Source: three-view drawing plus pictorial views. Frame: mm from the lowest corner of the part. A direction names the side the tool comes from. Give positions to 0.01 mm unless a question says otherwise; leave off trailing zeros. Loops run counter-clockwise (first coordinate to the right, second up) from the corner with the lowest first, then second, coordinate; pieces in that order, holes last. Notation, with made-up numbers: (23.25, -33) - (63.25, -33) arc R29 ccw to (63.25, -8) - close; hole circle Ø7 at (-30, -7.75). An arc over 180 degrees is marked (long way). Answer as a JSON object with one key per item and string values.
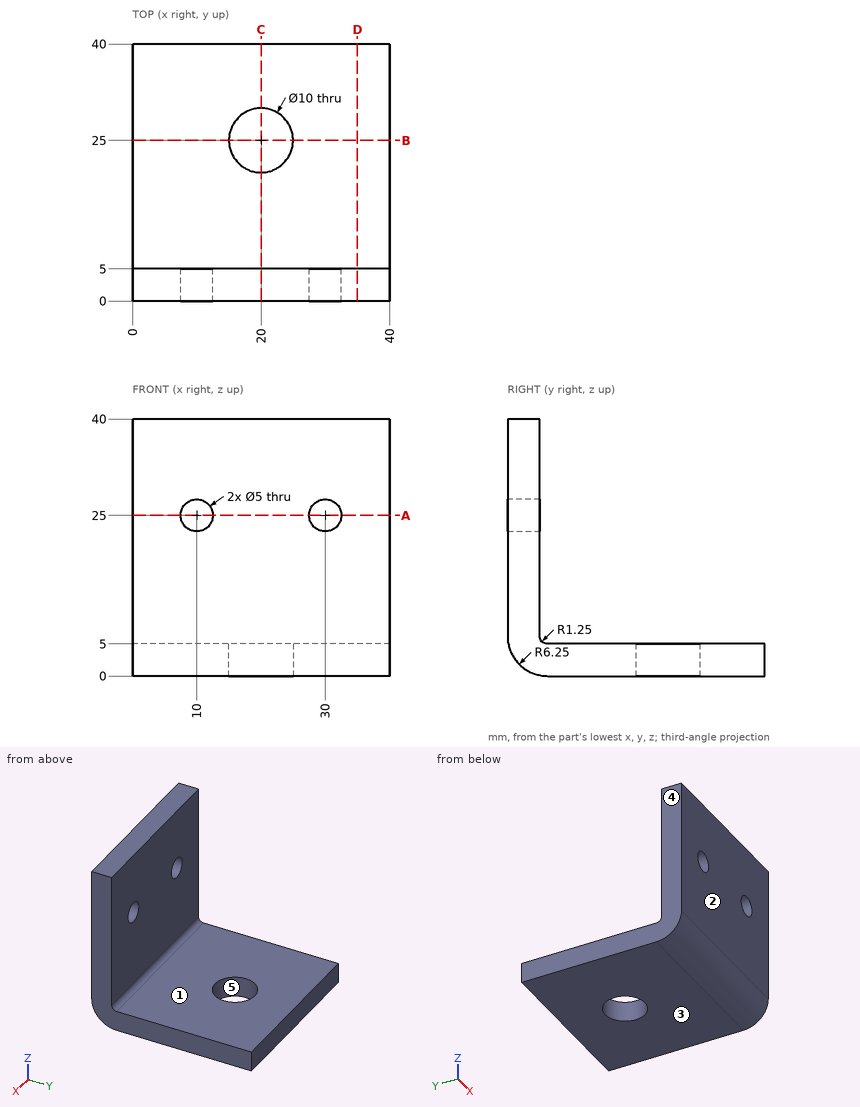
Item 1: Contact query for flat-ended pins moving along their axis: P1, Ø12, axis at x = 22.5, y = 18.5, coming from the +Z side; P2, Ø1.5, axis at x = 28.5, z = 29.5, coming from the +Y side; P3, Ø1, axis at x = 5.5, y = 23, coming from the -Z side. Output: stop coordinate, or through.
Geometry check:
{"P1": "stops at z = 5", "P2": "stops at y = 5", "P3": "stops at z = 0"}
Item 2: Cut plane B-B (y = 25). Return loops of the section in (x, z).
Geometry check:
{"outline": "(0, 0) - (15, 0) - (15, 5) - (0, 5) - close; (25, 0) - (40, 0) - (40, 5) - (25, 5) - close"}
Item 3: Material intervals for line 1 (X direction, y = 1, z = 25); line 2 (Y direction, x = 35, z = 24), sorted ascending. Write a range as [from, to].
Geometry check:
{"line 1": "x = [0, 7.5], [12.5, 27.5], [32.5, 40]", "line 2": "y = [0, 5]"}
Item 4: Cut plane D-D (x = 35). Return loops of the section in (y, z), then the cut area to 3 significant figures.
Geometry check:
{"outline": "(0, 6.25) arc R6.25 ccw to (6.25, 0) - (40, 0) - (40, 5) - (6.25, 5) arc R1.25 cw to (5, 6.25) - (5, 40) - (0, 40) - close", "area": "367 mm2"}
Item 5: Cut plane C-C (x = 20). Return loops of the section in (y, z), then the cut area to 3 significant figures.
Geometry check:
{"outline": "(0, 6.25) arc R6.25 ccw to (6.25, 0) - (20, 0) - (20, 5) - (6.25, 5) arc R1.25 cw to (5, 6.25) - (5, 40) - (0, 40) - close; (30, 0) - (40, 0) - (40, 5) - (30, 5) - close", "area": "317 mm2"}
Item 6: Cut plane A-A (z = 25). Return loops of the section in (x, y).
Geometry check:
{"outline": "(0, 0) - (7.5, 0) - (7.5, 5) - (0, 5) - close; (12.5, 0) - (27.5, 0) - (27.5, 5) - (12.5, 5) - close; (32.5, 0) - (40, 0) - (40, 5) - (32.5, 5) - close"}
Item 7: Access query for the marked faces 1 and 2. Directions: +Z, -Z, +X, -X, +Y, -Y. A direction counts if a zero-diameter tool reaches every point of the face in a straight line with its end or side. Return the directions, or none.
Geometry check:
{"face 1": "+Z, +X, -X, +Y", "face 2": "+Z, -Z, +X, -X, -Y"}
Item 8: Mould query, pull axis X, two halves, no side actions, for the marked faces 3, 4 and 5. Classes: released by +X, released by -X, zero draft, split by the parting line, or undercut.
Geometry check:
{"face 3": "zero draft", "face 4": "released by -X", "face 5": "undercut"}
